```python
from build123d import *

# Parameters (mm, degrees)
SKETCH1_R           = 57.5
BOSS_EXTRUDE1_DEPTH = 2.5


with BuildPart() as part:
    # Sketch1 → Boss-Extrude1 (new body)
    with BuildSketch(Plane.XY):
        with BuildLine():
            Line((-200, 0), (200, 0))
            Line((200, 0), (200, 2510.325909419))
            ThreePointArc((200, 2510.325909419), (0, 2517), (-200, 2510.325909419))
            Line((-200, 2510.325909419), (-200, 0))
        make_face()
        with Locations((0, 2020)):
            Circle(SKETCH1_R, mode=Mode.SUBTRACT)
        with Locations((0, 1140)):
            Circle(SKETCH1_R, mode=Mode.SUBTRACT)
    extrude(amount=BOSS_EXTRUDE1_DEPTH)


solid = part.part
```
Design review of the part built by this model. Coordinates are the model's own, in mm. Coordinates: 2 decimals unless noted, no trailing zeros. Loops run counter-clockwise (first coordinate to the right, second up) from the corner with the lowest first, then second, coordinate; pieces in that order, holes last. Notation, with made-up numbers: (76.5, 51) - (111.5, 51) arc R3 cw to (111.5, 55) - close; hole circle Ø11 at (5.5, 33). An arc over 180 degrees is marked (long way). Use CSV: the item, a comma, the result in double quotes. Start each with the question number.
1) Consider section B-B on x = 0. Write out the cut boundary in (y, z).
2) The part is to be moulded in two halves that separate along Y. For faces 1 (the flat face through (-3, 1276, 2.5)), 2 (the cylindrical face through (30.912, 2068.484, 1.232)), say which applies: +Y half, -Y half, draft (parallel to the pull), parting line (faces both ways), or undercut.
3) Consider section C-C on z = 0.55. Write out the cut boundary in (x, y).
4) Wall thickness on L1, parallel to Y at x = 0, z = 0.75; L2, parallel to Y at x = -4, z = 2.3; L3, parallel to X at y = 1983.5, z = 0.15: over which ranges is each line inside the solid? List them lowest first. Write a range as from..to.
5) Consider section A-A on y = 2020. Write out the cut boundary in (x, z), then the cut area to 4 significant figures.
Geometry says:
1,outline,"(0, 0) - (1082.5, 0) - (1082.5, 2.5) - (0, 2.5) - close; (1197.5, 0) - (1962.5, 0) - (1962.5, 2.5) - (1197.5, 2.5) - close; (2077.5, 0) - (2517, 0) - (2517, 2.5) - (2077.5, 2.5) - close"
2,face 1,"draft"
2,face 2,"undercut"
3,outline,"(-200, 0) - (200, 0) - (200, 2510.33) arc R3000 ccw to (-200, 2510.33) - close; hole circle Ø115 at (0, 1140); hole circle Ø115 at (0, 2020)"
4,L1,"0..1082.5, 1197.5..1962.5, 2077.5..2517"
4,L2,"0..1082.64, 1197.36..1962.64, 2077.36..2517"
4,L3,"-200..-44.43, 44.43..200"
5,outline,"(-200, 0) - (-57.5, 0) - (-57.5, 2.5) - (-200, 2.5) - close; (57.5, 0) - (200, 0) - (200, 2.5) - (57.5, 2.5) - close"
5,area,"712.5 mm^2"
